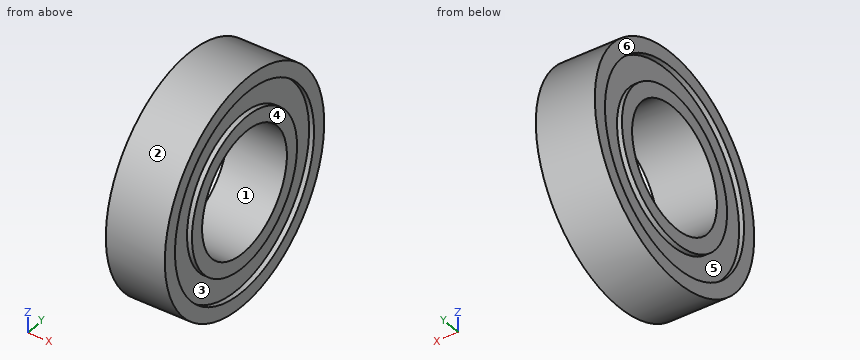
```python
from build123d import *


with BuildPart() as part:
    # Sketch1 → Revolve1 (revolve)
    with BuildSketch(Plane.XY, mode=Mode.PRIVATE) as revolve1_sk:
        Polygon((13.120246846, 20.5), (13.120246846, 23.5), (25.120246846, 23.5), (25.120246846, 20.5), (24.120246846, 20.5), (24.120246846, 15.5), (25.120246846, 15.5), (25.120246846, 12.5), (13.120246846, 12.5), (13.120246846, 15.5), (14.120246846, 15.5), (14.120246846, 20.5), align=None)
    revolve(revolve1_sk.sketch.rotate(Axis((0, 0, 0), (1, 0, 0)), 90), axis=Axis((0, 0, 0), (1, 0, 0)))


solid = part.part
```
The listing builds one solid part. Answer for the finished solid, in the listing's coordinates (mm). Face numbers are marked on the shaded views. A direction names the side the tool comes from. Coordinates: 2 decimals unless noted, no trailing zeros. Write each loop counter-clockwise with the first axis right and the second up, starting at its lowest first coordinate (ties: lowest second). Pieces come first, ordered by that corner, then holes. Notation, with made-up numbers: (88, -29) - (110, -29) arc R22 ccw to (110, -19) - close; hole circle Ø9 at (-16.5, 59). An arc over 180 degrees is marked (long way). Return JSON: item names as keys, results as strings. Group by question number.
1. A cutting plane is placed at C-C, the plane x = 20.75. Determine the outline of the cut face in (y, z).
2. Given pin 1 (1.5 mm diameter, centred on x = 15.5, y = -16, fed in from -Z); pin 2 (24.5 mm diameter, centred on y = 0, z = 0, fed in from -X) (1 decimal); pin 3 (1.5 mm diameter, centred on x = 21, z = -12.5, fed in from -Y); pin 4 (2 mm diameter, centred on x = 16, z = -5.5, fed in from +Y), each flat-ended and moving along its own axis, determine where each tip first touches the part or whether it passes through.
3. Which of the six approach directions +Z, -Z, +X, -X, +Y, -Y give full straight-line access (tool end or side, diameter ignored) to the marked faces 5 and 6?
4. Determine the mould class of the marked faces 1, 2, 3 and 4 for opening direction Z: released by +Z, released by -Z, zero draft, split by the parting line, or undercut.
5. A cutting plane is placed at D-D, the plane z = -17.5. Determine the outline of the cut face in (x, y), plus the area to 3 significant figures.
6. A cutting plane is placed at A-A, the plane z = 0. Determine the outline of the cut face in (x, y).
7. Straight lines are drawn through the part: L1, parallel to Y at x = 13.5, z = 0; L2, parallel to Y at x = 15.75, z = 0; L3, parallel to Z at x = 17.5, y = 9. For each, find the intervals that lie inside material, in ascending order.
Ans:
{
 "1": {"outline": "circle Ø47 at (0, 0); hole circle Ø25 at (0, 0)"},
 "2": {"pin 1": "z = -17.88", "pin 2": "through", "pin 3": "y = -20.35", "pin 4": "y = 23.07"},
 "3": {"face 5": "-X", "face 6": "+Z, -Z, -X, +Y, -Y"},
 "4": {"face 1": "undercut", "face 2": "split by the parting line", "face 3": "undercut", "face 4": "zero draft"},
 "5": {"outline": "(13.12, -15.68) - (25.12, -15.68) - (25.12, -10.68) - (24.12, -10.68) - (24.12, 10.68) - (25.12, 10.68) - (25.12, 15.68) - (13.12, 15.68) - (13.12, 10.68) - (14.12, 10.68) - (14.12, -10.68) - (13.12, -10.68) - close", "area": "334 mm²"},
 "6": {"outline": "(13.12, -23.5) - (25.12, -23.5) - (25.12, -20.5) - (24.12, -20.5) - (24.12, -15.5) - (25.12, -15.5) - (25.12, -12.5) - (13.12, -12.5) - (13.12, -15.5) - (14.12, -15.5) - (14.12, -20.5) - (13.12, -20.5) - close; (13.12, 12.5) - (25.12, 12.5) - (25.12, 15.5) - (24.12, 15.5) - (24.12, 20.5) - (25.12, 20.5) - (25.12, 23.5) - (13.12, 23.5) - (13.12, 20.5) - (14.12, 20.5) - (14.12, 15.5) - (13.12, 15.5) - close"},
 "7": {"L1": "-23.5 to -20.5, -15.5 to -12.5, 12.5 to 15.5, 20.5 to 23.5", "L2": "-23.5 to -12.5, 12.5 to 23.5", "L3": "-21.71 to -8.67, 8.67 to 21.71"}
}
